```python
from build123d import *

# Parameters (mm, degrees)
SKETCH_1_R              = 15
EXTRUDE_1_DEPTH         = 160
CHAMFER_1_SIZE          = 0.5
HOLE_WIZARD_M10_2_D     = 8.5
HOLE_WIZARD_M10_2_DEPTH = 24.5
HOLE_WIZARD_M10_2_TIP   = 2.553657631
HOLE_WIZARD_M10_1_D     = 8.5
HOLE_WIZARD_M10_1_DEPTH = 24.5
HOLE_WIZARD_M10_1_TIP   = 2.553657631


with BuildPart() as part:
    # 草图1 → 凸台-拉伸1 (new, symmetric)
    with BuildSketch(Plane(origin=(0, 0, 0), x_dir=(1, 0, 0), z_dir=(0, 1, 0))):
        with Locations(Location((0, 0, 0), (0, 0, 270))):
            Circle(SKETCH_1_R)
    extrude(amount=EXTRUDE_1_DEPTH, both=True)

    # 倒角1
    chamfer_1_edges = [part.edges().sort_by_distance(p)[0] for p in [
        (0, -160, -15),
        (0, 160, -15),
    ]]
    chamfer(chamfer_1_edges, length=CHAMFER_1_SIZE)

    # M10 螺纹孔2
    with Locations(Plane(origin=(0, 160, 0), x_dir=(1, 0, 0), z_dir=(0, 1, 0))):
        with Locations((0, 0)):
            Hole(HOLE_WIZARD_M10_2_D / 2, depth=HOLE_WIZARD_M10_2_DEPTH)
            with Locations((0, 0, -(HOLE_WIZARD_M10_2_DEPTH + HOLE_WIZARD_M10_2_TIP / 2))):  # 118° drill point
                Cone(0, HOLE_WIZARD_M10_2_D / 2, HOLE_WIZARD_M10_2_TIP, mode=Mode.SUBTRACT)

    # M10 螺纹孔1
    with Locations(Plane(origin=(0, -160, 0), x_dir=(-1, 0, 0), z_dir=(0, -1, 0))):
        with Locations((0, 0)):
            Hole(HOLE_WIZARD_M10_1_D / 2, depth=HOLE_WIZARD_M10_1_DEPTH)
            with Locations((0, 0, -(HOLE_WIZARD_M10_1_DEPTH + HOLE_WIZARD_M10_1_TIP / 2))):  # 118° drill point
                Cone(0, HOLE_WIZARD_M10_1_D / 2, HOLE_WIZARD_M10_1_TIP, mode=Mode.SUBTRACT)


solid = part.part
```
Build history of the part. All positions in model axes, mm. A direction names the side the tool comes from. Round coordinates to 2 decimals unless told otherwise and drop trailing zeros. Order: outer loops, then holes, each group sorted by start corner. A loop starts at its lowest first (then second) coordinate and runs counter-clockwise, first axis right, second up. Notation, with made-up numbers: (-3, -17) -> (6, -17) arc R18 ccw to (6, 4) -> close; hole circle Ø5 at (-14.75, 54). An arc over 180 degrees is marked (long way). Answer in a Markdown table with one row per item.
1) Band-saw the part on A-A on y = 53. Give the cut face in (x, z), and give its area (3 significant figures).
Values:
| item | result |
|---|---|
| outline | circle Ø30 at (0, 0) |
| area | 707 mm2 |
2) Wall check: L1, parallel to Z at x = 3.75, y = 27; L2, parallel to Z at x = -3.75, y = 140.5; L3, parallel to Z at x = -0.5, y = 128. Give the ranges that are in metal, low to high.
Values:
| item | result |
|---|---|
| L1 | -14.52 to 14.52 |
| L2 | -14.52 to -2, 2 to 14.52 |
| L3 | -14.99 to 14.99 |
3) Mould opens along Z. For faces 1 (the flat face through (3.4, 160, 3)), 2 (the conical face through (0.16, -133.39, 0.72)), 3 (the cylindrical face through (0.66, 2.233, -14.985)) say: released by +Z, released by -Z, zero draft, split by the parting line, or undercut.
Values:
| item | result |
|---|---|
| face 1 | zero draft |
| face 2 | undercut |
| face 3 | split by the parting line |
4) Pin check, flat tips, straight feed: P1, Ø10, axis at x = -11.5, y = 20.5, coming from the -Z side; P2, Ø6, axis at y = 53, z = -10.5, coming from the +X side; P3, Ø1, axis at y = -86.5, z = 1, coming from the -X side. Stop position of each tip, or through.
Values:
| item | result |
|---|---|
| P1 | z = -13.52 |
| P2 | x = 12.99 |
| P3 | x = -14.99 |
5) Which spindle directions (+Z, -Z, +X, -X, +Y, -Y) get a long thin tool onto all of the face, cutting with end or side? Do faces 4 (the cylindrical face through (-2.285, 147.578, -3.584)), 5 (the flat face through (3.4, -160, 3)), 6 (the cylindrical face through (2.285, -147.578, -3.584)). Say none if no direction does.
Values:
| item | result |
|---|---|
| face 4 | +Y |
| face 5 | +Z, -Z, +X, -X, -Y |
| face 6 | -Y |
